Input: part model. Units: mm. Frame: model coordinates. Face numbers are marked on the shaded views. A direction names the side the tool comes from. Round coordinates to 2 decimals unless told otherwise and drop trailing zeros. Loops run counter-clockwise (first coordinate to the right, second up) from the corner with the lowest first, then second, coordinate; pieces in that order, holes last. Notation, with made-up numbers: (22, 46.25) -> (46, 46.25) arc R15 cw to (46, 72.25) -> close; hole circle Ø5 at (27, 37). An arc over 180 degrees is marked (long way). Answer as a JSON object with one key per item and string values. Group by question number.
Item 1: Section query B-B on x = 70.5. Return loops of the section in (y, z), and give its area (3 significant figures).
Item 2: Draft query along X for the marked faces 6, 7, 8 and 9. Return one class per face: released by +X, released by -X, zero draft, split by the parting line, or undercut.
Item 3: Material intervals for line 1 (X direction, y = -5, z = 28); line 2 (X direction, y = -113, z = -6.5); line 3 (Z direction, x = -6.5, y = -41), sorted ascending. Write a range as [from, to].
Item 4: Pin query (flat end, axial travel): pin 1 (8 mm diameter, centred on x = 87.5, z = 28.5, fed in from -Y); pin 2 (4.5 mm diameter, centred on y = -101.5, z = -43.5, fed in from +X); pin 3 (23 mm diameter, centred on x = 52.5, z = -24.5, fed in from -Y); pin 4 (6.5 mm diameter, centred on y = -11, z = 22.5, fed in from -X). Return the tip coordinate at first contact, or that it passes through.
Item 5: Section query D-D on z = -11. Return loops of the section in (x, y).
Item 6: Set-up query: the marked faces 1, 2, 3, 4 and 5. Return all of +Z, -Z, +X, -X, +Y, -Y with unobstructed straight access to the full face (end or side cutting, diameter ignored); none if empty.
Item 7: Section query A-A on y = -114. Return loops of the section in (x, z), and give its area (3 significant figures).
Item 8: Section query C-C on x = 8. Return loops of the section in (y, z).
from build123d import *

# Parameters (mm, degrees)
BASE_PLATE_DEPTH         = 15
LONG_SLOT_DEPTH          = 15
LOWER_BLOCK_SKETCH_W     = 66
LOWER_BLOCK_SKETCH_H     = 33
LOWER_BLOCK_33X66_DEPTH  = 15
BLOCK_EXTENSION_SKETCH_W = 29
BLOCK_EXTENSION_SKETCH_H = 9
BLOCK_EXTENSION_DEPTH    = 50
BLOCK_END_SKETCH_W       = 50
BLOCK_END_SKETCH_H       = 33
BLOCK_END_50X50_DEPTH    = 15
LUG_A_DEPTH              = 16
LUG_B_DEPTH              = 16
LUG_HOLES_SKETCH_R       = 2.5
LUG_HOLES_2X5MM_DEPTH    = 16


with BuildPart() as part:
    # Base Plate Profile Sketch → Base Plate (new body)
    with BuildSketch(Plane.XY):
        with BuildLine():
            Line((49, 0), (0, 0))
            Line((0, 0), (0, -19.125314072))
            ThreePointArc((0, -19.125314072), (-1.808661059, -23.821056825), (-6.3, -26.090226132))
            ThreePointArc((-6.3, -26.090226132), (-22.477429316, -44.901129951), (-4.5, -62))
            ThreePointArc((-4.5, -62), (-3.335967318, -61.893154357), (-2.167902709, -61.848286255))
            ThreePointArc((-2.167902709, -61.848286255), (14.519311725, -69.135443097), (20, -86.5))
            Line((20, -86.5), (20, -132))
            Line((20, -132), (34, -132))
            Line((34, -132), (34, -108))
            Line((34, -108), (64, -108))
            Line((64, -108), (64, -132))
            Line((64, -132), (78, -132))
            Line((78, -132), (78, -86.5))
            ThreePointArc((78, -86.5), (85.175883861, -69.175883861), (102.5, -62))
            ThreePointArc((102.5, -62), (120.477429316, -44.901129951), (104.3, -26.090226132))
            ThreePointArc((104.3, -26.090226132), (99.808661059, -23.821056825), (98, -19.125314072))
            Line((98, -19.125314072), (98, 0))
            Line((98, 0), (49, 0))
        make_face()
    extrude(amount=BASE_PLATE_DEPTH)

    # Long Slot Sketch → Long Slot (cut)
    with BuildSketch(Plane.XY.offset(15)):
        with BuildLine():
            Line((-4.5, -40.5), (102.5, -40.5))
            ThreePointArc((102.5, -40.5), (106, -44), (102.5, -47.5))
            Line((102.5, -47.5), (-4.5, -47.5))
            ThreePointArc((-4.5, -47.5), (-8, -44), (-4.5, -40.5))
        make_face()
    extrude(amount=-LONG_SLOT_DEPTH, mode=Mode.SUBTRACT)

    # Lower Block Sketch → Lower Block 33x66 (add)
    with BuildSketch(Plane.ZY.offset(-20)):
        with Locations((-18, -115.5)):
            Rectangle(LOWER_BLOCK_SKETCH_W, LOWER_BLOCK_SKETCH_H)
    extrude(amount=-LOWER_BLOCK_33X66_DEPTH)

    # Block Extension Sketch → Block Extension (add)
    with BuildSketch(Plane(origin=(0, 0, 0), x_dir=(-1, 0, 0), z_dir=(0, 0, -1))):
        with Locations((-49.5, -103.5)):
            Rectangle(BLOCK_EXTENSION_SKETCH_W, BLOCK_EXTENSION_SKETCH_H)
    extrude(amount=BLOCK_EXTENSION_DEPTH)

    # Block End Sketch → Block End 50x50 (add)
    with BuildSketch(Plane(origin=(78, 0, 0), x_dir=(0, 0, -1), z_dir=(1, 0, 0))):
        with Locations((10, -115.5)):
            Rectangle(BLOCK_END_SKETCH_W, BLOCK_END_SKETCH_H)
    extrude(amount=-BLOCK_END_50X50_DEPTH)

    # Lug A Sketch → Lug A (add)
    with BuildSketch(Plane(origin=(0, 0, 0), x_dir=(1, 0, 0), z_dir=(0, 1, 0))):
        with BuildLine():
            Line((8, -15), (0, -15))
            Line((0, -15), (0, -28))
            ThreePointArc((0, -28), (8, -36), (16, -28))
            Line((16, -28), (16, -15))
            Line((16, -15), (8, -15))
        make_face()
    extrude(amount=-LUG_A_DEPTH)

    # Lug B Sketch → Lug B (add)
    with BuildSketch(Plane(origin=(0, 0, 0), x_dir=(1, 0, 0), z_dir=(0, 1, 0))):
        with BuildLine():
            Line((98, -28), (98, -15))
            Line((98, -15), (90, -15))
            Line((90, -15), (82, -15))
            Line((82, -15), (82, -28))
            ThreePointArc((82, -28), (90, -36), (98, -28))
        make_face()
    extrude(amount=-LUG_B_DEPTH)

    # Lug Holes Sketch → Lug Holes 2x5mm (cut)
    with BuildSketch(Plane.XZ.offset(16)):
        with Locations(Location((90, 28, 0), (0, 0, 270))):
            Circle(LUG_HOLES_SKETCH_R)
        with Locations(Location((8, 28, 0), (0, 0, 270))):
            Circle(LUG_HOLES_SKETCH_R)
    extrude(amount=-LUG_HOLES_2X5MM_DEPTH, mode=Mode.SUBTRACT)


solid = part.part
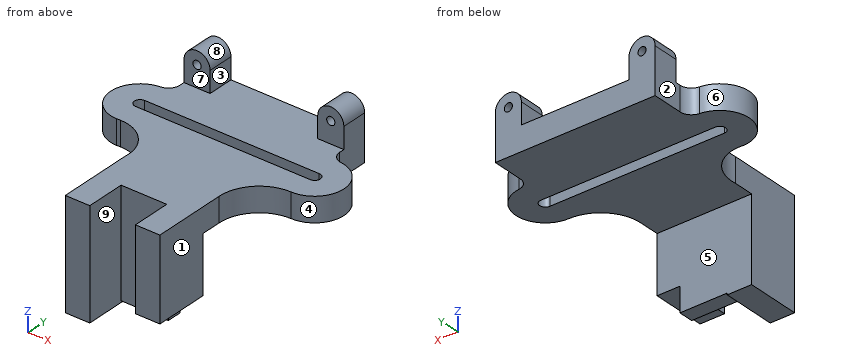
Solved:
{
 "1": {"outline": "(-132, -35) -> (-99, -35) -> (-99, 0) -> (-47.5, 0) -> (-47.5, 15) -> (-132, 15) -> close; (-40.5, 0) -> (0, 0) -> (0, 15) -> (-40.5, 15) -> close", "area": "3,030 mm²"},
 "2": {"face 6": "released by -X", "face 7": "zero draft", "face 8": "undercut", "face 9": "undercut"},
 "3": {"line 1": "[0, 5.5], [10.5, 16], [82, 87.5], [92.5, 98]", "line 2": "[20, 35], [63, 78]", "line 3": "[0, 15]"},
 "4": {"pin 1": "y = -16", "pin 2": "x = 64", "pin 3": "y = -132", "pin 4": "x = 0"},
 "5": {"outline": "(20, -132) -> (35, -132) -> (35, -108) -> (63, -108) -> (63, -132) -> (78, -132) -> (78, -99) -> (20, -99) -> close"},
 "6": {"face 1": "+Z, -Z, +X, -Y", "face 2": "+Z, -Z, -X, +Y", "face 3": "+Z, +Y, -Y", "face 4": "+Z, -Z, +X", "face 5": "-Z, +X, -X, +Y"},
 "7": {"outline": "(20, -51) -> (35, -51) -> (35, 15) -> (20, 15) -> close; (63, -35) -> (78, -35) -> (78, 15) -> (63, 15) -> close", "area": "1,740 mm²"},
 "8": {"outline": "(-64.17, 0) -> (-47.5, 0) -> (-47.5, 15) -> (-64.17, 15) -> close; (-40.5, 0) -> (0, 0) -> (0, 25.5) -> (-16, 25.5) -> (-16, 15) -> (-40.5, 15) -> close; (-16, 30.5) -> (0, 30.5) -> (0, 36) -> (-16, 36) -> close"}
}
